Geometry: see drawing. Coordinates: mm, zero at the bounding-box minimum. Coordinates: 2 decimals unless noted, no trailing zeros. Loops run counter-clockwise (first coordinate to the right, second up) from the corner with the lowest first, then second, coordinate; pieces in that order, holes last. Notation, with made-up numbers: (-8, -2.75) - (45, -2.75) arc R33 cw to (45, 33.25) - close; hole circle Ø5 at (-5, -14.5). An arc over 180 degrees is marked (long way). Use a Markdown table: item, result. Add a question column.
1. Section query D-D on x = 46. Return the cut outline in (y, z).
2. Section query C-C on x = 32. Return the cut outline in (y, z).
3. Ray query, L1, parallel to Y at x = 25, z = 4; L2, parallel to X at y = 36, z = 5; L3, parallel to X at y = 26, z = 2.75. Return the intervals inside material, ascending. Write a range as [from, to].
4. Draft query along X for the marked faces 1, 2, 3 and 4. Return one class per face: released by +X, released by -X, zero draft, split by the parting line, or undercut.
5. Section query B-B on z = 16.75. Return the cut outline in (x, y), then the cut area to 3 significant figures.
6. Section query A-A on y = 30. Return the cut outline in (x, z).
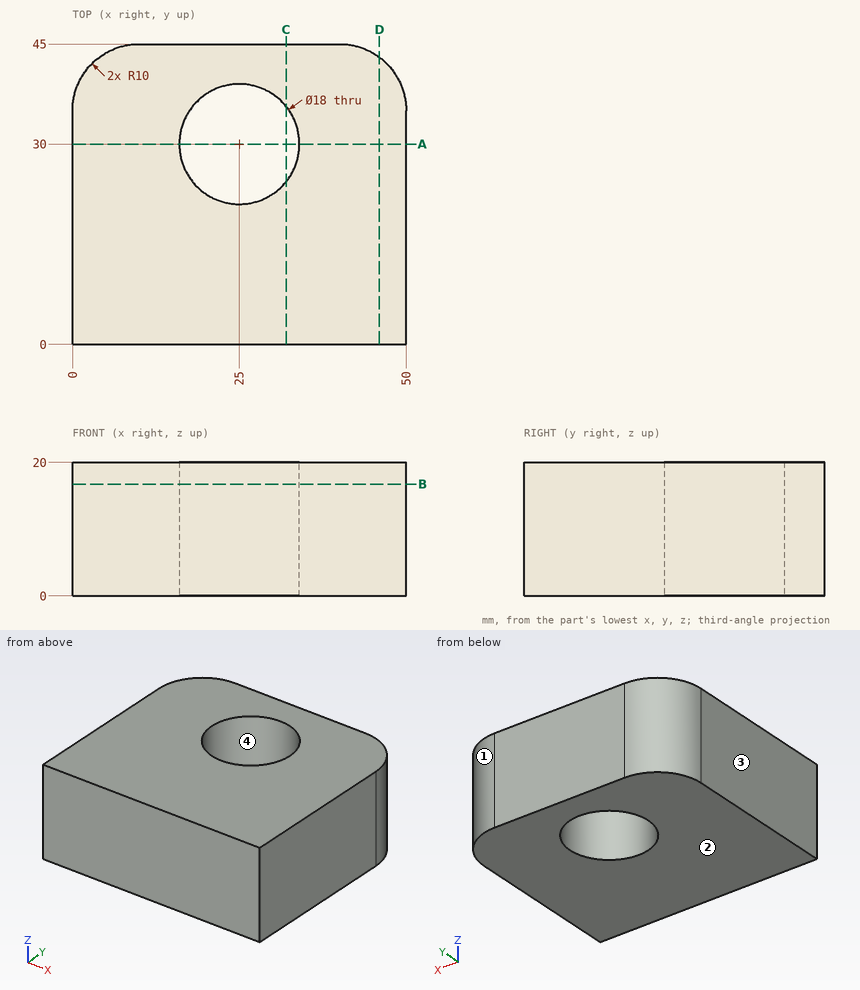
Resolved:
| question | item | result |
|---|---|---|
| 1 | outline | (0, 0) - (43, 0) - (43, 20) - (0, 20) - close |
| 2 | outline | (0, 0) - (24.34, 0) - (24.34, 20) - (0, 20) - close; (35.66, 0) - (45, 0) - (45, 20) - (35.66, 20) - close |
| 3 | L1 | [0, 21], [39, 45] |
| 3 | L2 | [0.05, 18.29], [31.71, 49.95] |
| 3 | L3 | [0, 16.94], [33.06, 50] |
| 4 | face 1 | released by +X |
| 4 | face 2 | zero draft |
| 4 | face 3 | released by -X |
| 4 | face 4 | undercut |
| 5 | outline | (0, 0) - (50, 0) - (50, 35) arc R10 ccw to (40, 45) - (10, 45) arc R10 ccw to (0, 35) - close; hole circle Ø18 at (25, 30) |
| 5 | area | 1,950 mm² |
| 6 | outline | (0, 0) - (16, 0) - (16, 20) - (0, 20) - close; (34, 0) - (50, 0) - (50, 20) - (34, 20) - close |
